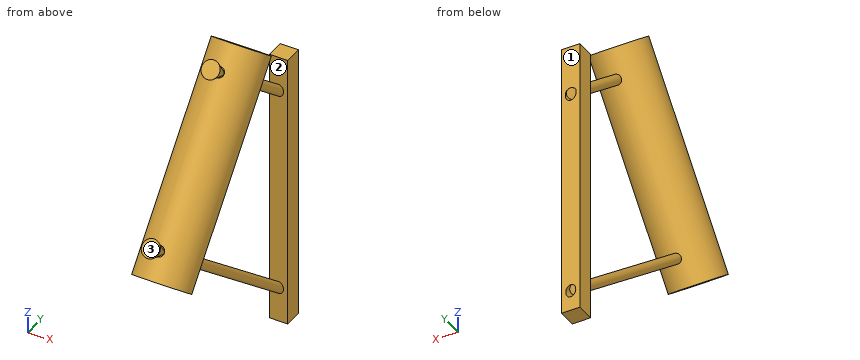
from build123d import *

# Parameters (mm, degrees)
SKETCH2_W                     = 15
SKETCH2_H                     = 230
BOSS_EXTRUDE2_DEPTH           = 15
SKETCH4_R                     = 4
BOSS_EXTRUDE3_DEPTH           = 155
SKETCH5_R                     = 4.473763718
CUT_EXTRUDE1_DEPTH            = 120
SKETCH6_R                     = 4.1
CUT_EXTRUDE2_DEPTH            = 17
SKETCH7_R                     = 5.311376806
SKETCH7_R_2                   = 5.6699774
CUT_EXTRUDE3_DEPTH            = 62
SKETCH8_R                     = 22.5
BOSS_EXTRUDE4_DEPTH           = 178
SKETCH9_R                     = 4.2
CUT_EXTRUDE4_DEPTH            = 8
SKETCH10_R                    = 2
BOSS_EXTRUDE5_DEPTH           = 20
BOSS_EXTRUDE5_DRAFT           = -15
BOSS_EXTRUDE5_PROFILE_2_DEPTH = 20
BOSS_EXTRUDE5_PROFILE_2_DRAFT = -15
SKETCH11_R                    = 15
CUT_EXTRUDE5_DEPTH            = 193


with BuildPart() as part:
    # Sketch2 → Boss-Extrude2 (new body)
    with BuildSketch(Plane(origin=(0, 0, 0), x_dir=(1, 0, 0), z_dir=(0, 1, 0))):
        with Locations((-7.5, -115)):
            Rectangle(SKETCH2_W, SKETCH2_H)
    extrude(amount=BOSS_EXTRUDE2_DEPTH)

    # Sketch4 → Boss-Extrude3 (add, symmetric)
    with BuildSketch(Plane(origin=(0, -112.486974084, 91.090155556), x_dir=(1, 0, 0), z_dir=(0, 0.7771459614569742, -0.6293203910498333))):
        with Locations(Location((-7.5, -22.665437835, 0), (0, 0, 270))):
            Circle(SKETCH4_R)
        with Locations(Location((-7.5, -156.375872868, 0), (0, 0, 270))):
            Circle(SKETCH4_R)
    extrude(amount=BOSS_EXTRUDE3_DEPTH, both=True)

    # Sketch5 → Cut-Extrude1 (cut)
    with BuildSketch(Plane(origin=(0, 7.970649941, -6.454505057), x_dir=(1, 0, 0), z_dir=(0, 0.7771459614569743, -0.6293203910498333))):
        with Locations((-7.5, -156.375872868)):
            Circle(SKETCH5_R)
    extrude(amount=-CUT_EXTRUDE1_DEPTH, mode=Mode.SUBTRACT)

    # Sketch6 → Cut-Extrude2 (cut)
    with BuildSketch(Plane(origin=(0, 7.970649941, -6.454505057), x_dir=(1, 0, 0), z_dir=(0, 0.7771459614569743, -0.6293203910498333))):
        with Locations(Location((-7.5, -22.665437835, 0), (0, 0, 270))):
            Circle(SKETCH6_R)
    extrude(amount=-CUT_EXTRUDE2_DEPTH, mode=Mode.SUBTRACT)

    # Sketch7 → Cut-Extrude3 (cut)
    with BuildSketch(Plane(origin=(0, -232.94459811, 188.634816169), x_dir=(1, 0, 0), z_dir=(0, -0.7771459614569743, 0.6293203910498333))):
        with Locations((-7.5, 22.665437835)):
            Circle(SKETCH7_R)
        with Locations((-7.5, 156.375872868)):
            Circle(SKETCH7_R_2)
    extrude(amount=-CUT_EXTRUDE3_DEPTH, mode=Mode.SUBTRACT)

    # Sketch8 → Boss-Extrude4 (add)
    with BuildSketch(Plane(origin=(0, 112.486974084, 138.909844444), x_dir=(1, 0, 0), z_dir=(0, -0.6293203910498333, -0.7771459614569743))):
        with Locations(Location((-7.5, 212.198540139, 0), (0, 0, 270))):
            Circle(SKETCH8_R)
    extrude(amount=BOSS_EXTRUDE4_DEPTH)

    # Sketch9 → Cut-Extrude4 (cut)
    with BuildSketch(Plane(origin=(0, -184.7615485, 149.616951924), x_dir=(1, 0, 0), z_dir=(0, -0.7771459614569743, 0.6293203910498334))):
        with Locations(Location((-7.5, 156.375872868, 0), (0, 0, 270))):
            Circle(SKETCH9_R)
        with Locations(Location((-7.5, 22.665437835, 0), (0, 0, 270))):
            Circle(SKETCH9_R)
    extrude(amount=-CUT_EXTRUDE4_DEPTH, mode=Mode.SUBTRACT)


with BuildPart() as boss_extrude5_tool:
    # Sketch10 → Boss-Extrude5 (with draft: the straight prism first)
    with BuildSketch(Plane(origin=(0, -178.544380808, 144.582388795), x_dir=(1, 0, 0), z_dir=(0, -0.777145961456974, 0.6293203910498335))):
        with Locations((-7.5, 156.375872868)):
            Circle(SKETCH10_R)
    extrude(amount=BOSS_EXTRUDE5_DEPTH)
    # Boss-Extrude5: the draft: its side faces are tilted about the plane it starts from
    boss_extrude5_sides = [boss_extrude5_tool.faces().sort_by_distance(p)[0] for p in [
        (-9.5, -87.905314959, 272.402470774),
    ]]
    draft(boss_extrude5_sides, Plane(origin=(0, -178.544380808, 144.582388795), x_dir=(1, 0, 0), z_dir=(0, -0.777145961456974, 0.6293203910498335)), BOSS_EXTRUDE5_DRAFT)


with BuildPart() as part_1:
    add(part.part)

    # Boss-Extrude5: add boss_extrude5_tool
    add(boss_extrude5_tool.part)


with BuildPart() as boss_extrude5_profile_2_tool:
    # Sketch10 → Boss-Extrude5 profile 2 (with draft: the straight prism first)
    with BuildSketch(Plane(origin=(0, -178.544380808, 144.582388795), x_dir=(1, 0, 0), z_dir=(0, -0.777145961456974, 0.6293203910498335))):
        with Locations((-7.5, 22.665437835)):
            Circle(SKETCH10_R)
    extrude(amount=BOSS_EXTRUDE5_PROFILE_2_DEPTH)
    # Boss-Extrude5 profile 2: the draft: its side faces are tilted about the plane it starts from
    boss_extrude5_profile_2_sides = [boss_extrude5_profile_2_tool.faces().sort_by_distance(p)[0] for p in [
        (-9.5, -172.052018221, 168.489946184),
    ]]
    draft(boss_extrude5_profile_2_sides, Plane(origin=(0, -178.544380808, 144.582388795), x_dir=(1, 0, 0), z_dir=(0, -0.777145961456974, 0.6293203910498335)), BOSS_EXTRUDE5_PROFILE_2_DRAFT)


with BuildPart() as part_2:
    add(part_1.part)

    # Boss-Extrude5 profile 2: add boss_extrude5_profile_2_tool
    add(boss_extrude5_profile_2_tool.part)

    # Sketch11 → Cut-Extrude5 (cut)
    with BuildSketch(Plane(origin=(0, 112.486974084, 138.909844444), x_dir=(1, 0, 0), z_dir=(0, 0.6293203910498334, 0.7771459614569743))):
        with Locations(Location((-7.5, -212.198540139, 0), (0, 0, 270))):
            Circle(SKETCH11_R)
    extrude(amount=-CUT_EXTRUDE5_DEPTH, mode=Mode.SUBTRACT)


solid = part_2.part
Part model, mm, in its own coordinate system. Face numbers are marked on the shaded views. Round coordinates to 2 decimals unless told otherwise and drop trailing zeros. Loops run counter-clockwise (first coordinate to the right, second up) from the corner with the lowest first, then second, coordinate; pieces in that order, holes last. Notation, with made-up numbers: (-25, -23) - (-13, -23) arc R10 cw to (-13, -12) - close; hole circle Ø11 at (20, 1). An arc over 180 degrees is marked (long way). Answer as a JSON object with one key per item and string values.
Item 1: Wall check: L1, parallel to Z at x = -6.5, y = -101; L2, parallel to X at y = -83, z = 229.5; L3, parallel to Y at x = -8, z = 201. Give the ranges that are in metal, low to high.
Output:
{"L1": "105.97 to 115.94, 176.74 to 188.68, 236.24 to 248.18", "L2": "-29.76 to -22.14, 7.14 to 14.76", "L3": "-139.23 to -129.57, -90.99 to -81.34, -6.04 to 15"}
Item 2: Pin check, flat tips, straight feed: pin 1 (8 mm diameter, centred on x = -12, z = 111.5, fed in from +Y); pin 2 (8 mm diameter, centred on x = -20, y = -65, fed in from -Z); pin 3 (7.5 mm diameter, centred on x = -10, z = 149.5, fed in from -Y). Stop position of each tip, or through.
Output:
{"pin 1": "y = 15", "pin 2": "z = 221.01", "pin 3": "y = -181.93"}
Item 3: Pull direction Z, two halves, no side cores. Call the marked faces 1, 2 and 3: pulls with the +Z half, pulls with the -Z half, needs draft (parallel to the pull), parting line crosses it, or undercut.
Output:
{"face 1": "needs draft", "face 2": "undercut", "face 3": "pulls with the +Z half"}
Item 4: Band-saw the part on A-A on x = 4. List the corners of the cut face in (y, z).
Output:
{"outline": "(-179.47, 146.29) - (-171.93, 140.18) - (-59.91, 278.51) - (-67.45, 284.62) - close; (-156.96, 128.06) - (-149.41, 121.95) - (-37.39, 260.28) - (-44.94, 266.39) - close"}
